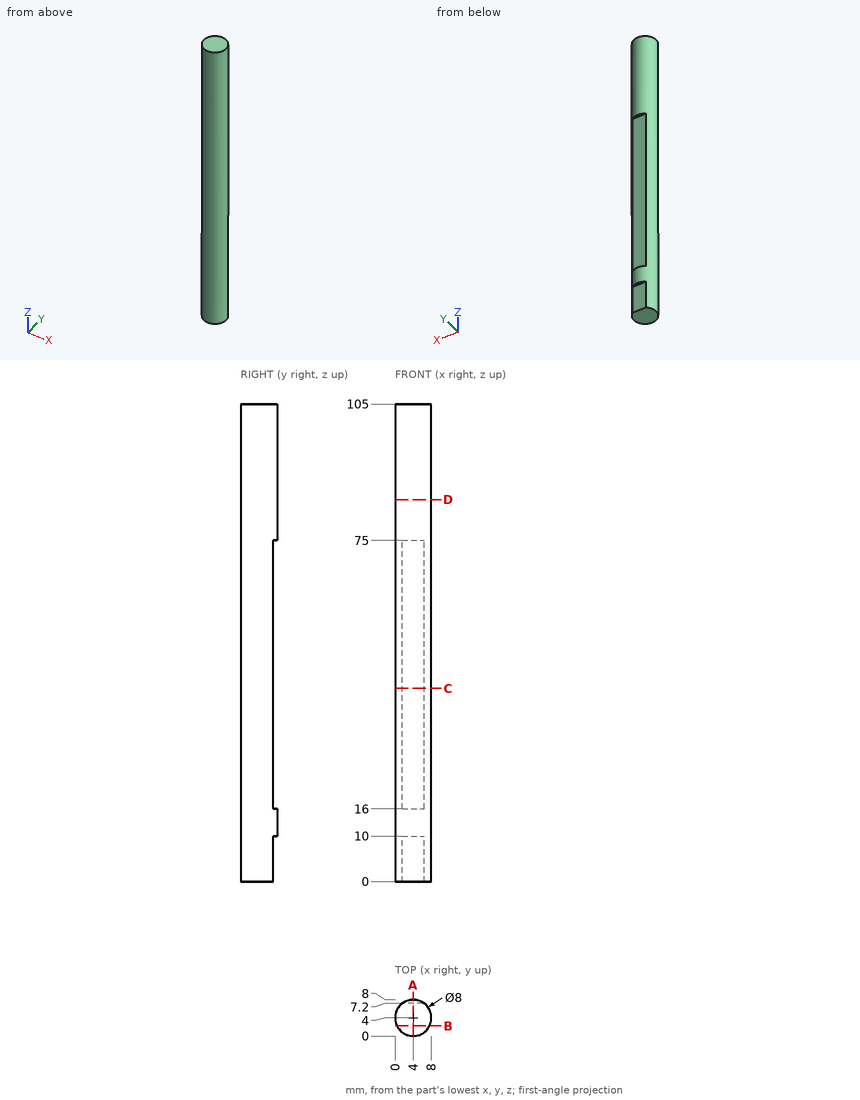
Can you work these out from the drawing? Everything is in mm from the part's minimum corner. Give positions to 0.01 mm unless a question says otherwise; leave off trailing zeros. Order: outer loops, then holes, each group sorted by start corner. A loop starts at its lowest first (then second) coordinate and runs counter-clockwise, first axis right, second up. Notation, with made-up numbers: M -30.5,52.25 L -18.5,52.25 A27 cw -18.5,71.25 Z; hole C -17,-9 d7. An arc over 180 degrees is marked long. Use a Markdown table: item, result. Add a question column.
Item 1: Suppose I cut it at D-D (z = 84). List the corners of the cut face in (x, y) for me, then the cut area to 3 significant figures.
Item 2: Suppose I cut it at C-C (z = 42.5). List the corners of the cut face in (x, y) for me.
Item 3: Suppose I cut it at B-B (y = 2.25). List the corners of the cut face in (x, z) for me, then the cut area to 3 significant figures.
Item 4: Suppose I cut it at A-A (x = 4). List the corners of the cut face in (y, z) for me, then the cut area to 3 significant figures.
Item 5: Will these pins go through, and if not, where does the flat tip stop? pin 1 (2.5 mm diameter, centred on x = 5, z = 60, fed in from +Y); pin 2 (2 mm diameter, centred on x = 2.5, z = 10.5, fed in from +Y).
Item 6: If I drill on L1, parallel to Z at x = 5, y = 7.5; L2, parallel to X at y = 3.75, z = 59.5; L3, parallel to Y at x = 6.25, z = 30.5, over which ranges is the centre line in solid material (lowest first)? Write a range as [from, to].
Answer sheet:
| question | item | result |
|---|---|---|
| 1 | outline | C 4,4 d8 |
| 1 | area | 50.3 mm² |
| 2 | outline | M 1.6,7.2 A4 ccw long 6.4,7.2 Z |
| 3 | outline | M 0.4,0 L 7.6,0 L 7.6,105 L 0.4,105 Z |
| 3 | area | 755 mm² |
| 4 | outline | M 0,0 L 7.2,0 L 7.2,10 L 8,10 L 8,16 L 7.2,16 L 7.2,75 L 8,75 L 8,105 L 0,105 Z |
| 4 | area | 785 mm² |
| 5 | pin 1 | stops at y = 7.2 |
| 5 | pin 2 | stops at y = 7.97 |
| 6 | L1 | z = [10, 16], [75, 105] |
| 6 | L2 | x = [0.01, 7.99] |
| 6 | L3 | y = [0.69, 7.2] |
